The figure shows three views and two pictorial views of one solid part (mm, origin at its lowest corner). Answer the questions. Coordinates: 2 decimals unless noted, no trailing zeros. Loops run counter-clockwise (first coordinate to the right, second up) from the corner with the lowest first, then second, coordinate; pieces in that order, holes last. Notation, with made-up numbers: (45.5, -11.5) - (80.5, -11.5) arc R9 ccw to (80.5, 5.5) - close; hole circle Ø2 at (-16, 26.5). An arc over 180 degrees is marked (long way). One line per question, with ' | ' between items.
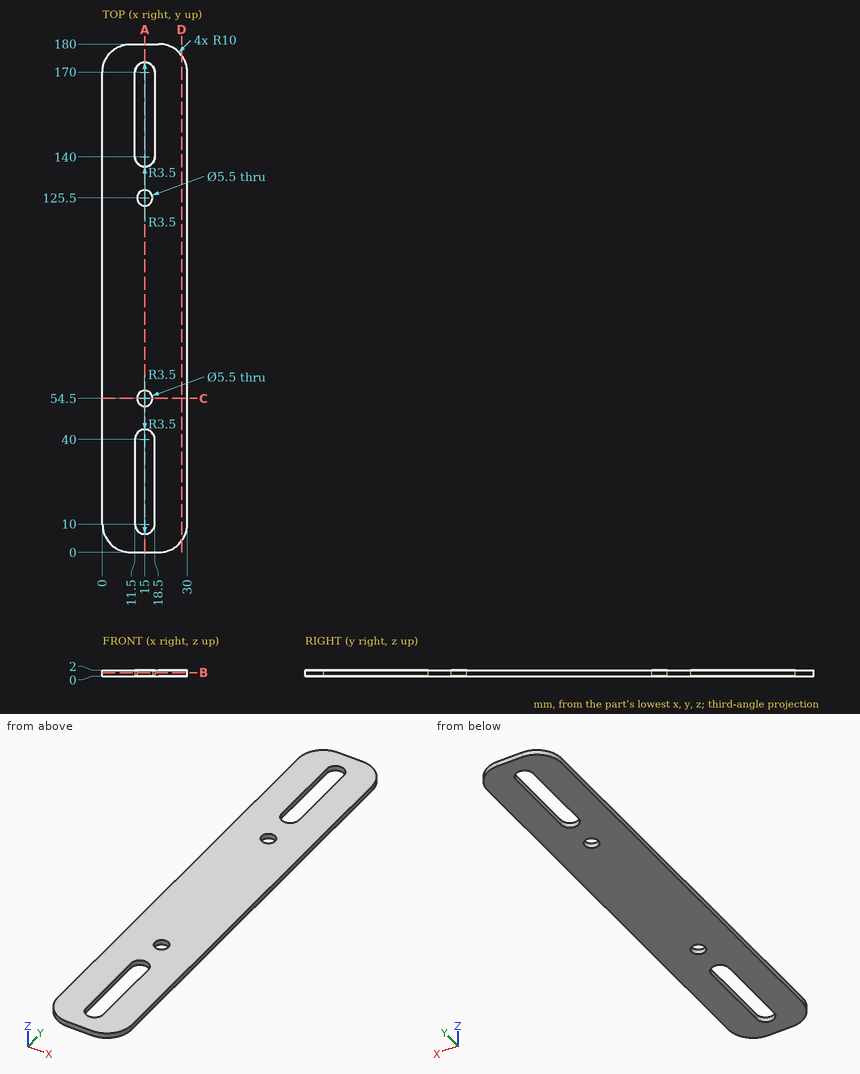
Item 1: Find section B-B, the plane z = 1.2. Write down the section's boundary in (x, y).
Taken from the geometry:
outline: (0, 10) arc R10 ccw to (10, 0) - (20, 0) arc R10 ccw to (30, 10) - (30, 170) arc R10 ccw to (20, 180) - (10, 180) arc R10 ccw to (0, 170) - close; hole (11.5, 10) arc R3.5 ccw to (18.5, 10) - (18.5, 40) arc R3.5 ccw to (11.5, 40) - close; hole (11.5, 140) arc R3.5 ccw to (18.5, 140) - (18.5, 170) arc R3.5 ccw to (11.5, 170) - close; hole circle Ø5.5 at (15, 54.5); hole circle Ø5.5 at (15, 125.5)
Item 2: Find section D-D, the plane x = 28. Write down the section's boundary in (y, z).
Taken from the geometry:
outline: (4, 0) - (176, 0) - (176, 2) - (4, 2) - close
Item 3: Find the intervals of material crossed by line 1 (Y direction, x = 15, z = 1.4); line 2 (X direction, y = 159, z = 0.8); line 3 (Y direction, x = 17, z = 0.75), in increasing order. Write a range as [from, to].
Taken from the geometry:
line 1: y = [0, 6.5], [43.5, 51.75], [57.25, 122.75], [128.25, 136.5], [173.5, 180] | line 2: x = [0, 11.5], [18.5, 30] | line 3: y = [0, 7.13], [42.87, 52.61], [56.39, 123.61], [127.39, 137.13], [172.87, 180]
Item 4: Find section C-C, the plane y = 54.5. Write down the section's boundary in (x, z).
Taken from the geometry:
outline: (0, 0) - (12.25, 0) - (12.25, 2) - (0, 2) - close; (17.75, 0) - (30, 0) - (30, 2) - (17.75, 2) - close
Item 5: Find section A-A, the plane x = 15. Write down the section's boundary in (y, z).
Taken from the geometry:
outline: (0, 0) - (6.5, 0) - (6.5, 2) - (0, 2) - close; (43.5, 0) - (51.75, 0) - (51.75, 2) - (43.5, 2) - close; (57.25, 0) - (122.75, 0) - (122.75, 2) - (57.25, 2) - close; (128.25, 0) - (136.5, 0) - (136.5, 2) - (128.25, 2) - close; (173.5, 0) - (180, 0) - (180, 2) - (173.5, 2) - close
